from build123d import *

# Parameters (mm, degrees)
CUT_EXTRUDE1_DEPTH = 2.54
FILLET2_R          = 0.8128


with BuildPart() as part:
    # Sketch1 → Revolve1 (revolve)
    with BuildSketch(Plane.XY):
        Polygon((0, 5.842), (0, 12.7), (-6.35, 12.7), (-6.35, 0), (0, 0), (127, 0), (127, 5.842), align=None)
    revolve(axis=Axis((127, 0, 0), (-1, 0, 0)))

    # Sketch2 → Cut-Extrude1 (cut)
    with BuildSketch(Plane.ZY.offset(6.35)):
        Polygon((-2.54, 6.35), (-2.54, 2.54), (-6.35, 2.54), (-6.35, -2.54), (-2.54, -2.54), (-2.54, -6.122575092), (2.54, -6.122575092), (2.54, -2.54), (6.35, -2.54), (6.35, 2.54), (2.54, 2.54), (2.54, 6.35), align=None)
    extrude(amount=-CUT_EXTRUDE1_DEPTH, mode=Mode.SUBTRACT)

    # Fillet2
    fillet2_edges = [part.edges().sort_by_distance(p)[0] for p in [
        (-6.35, 6.35, 0),
        (-6.35, 4.445, -2.54),
        (-6.35, 2.54, -4.445),
        (-6.35, 0, -6.35),
        (-6.35, -2.54, -4.445),
        (-6.35, -4.331287546, -2.54),
        (-6.35, -6.122575092, 0),
        (-6.35, -4.331287546, 2.54),
        (-6.35, -2.54, 4.445),
        (-6.35, 0, 6.35),
        (-6.35, 2.54, 4.445),
        (-6.35, 4.445, 2.54),
    ]]
    fillet(fillet2_edges, radius=FILLET2_R)


solid = part.part
Geometry check sheet. Reference: the model listing, model coordinates, mm. Coordinates: 2 decimals unless noted, no trailing zeros. Loops run counter-clockwise (first coordinate to the right, second up) from the corner with the lowest first, then second, coordinate; pieces in that order, holes last. Notation, with made-up numbers: (-25.75, 46.5) - (14.25, 46.5) arc R26 cw to (14.25, 67.5) - close; hole circle Ø1 at (88.25, -3). An arc over 180 degrees is marked (long way). Use one line per item in the form item = value. Start each with the question number.
Item 1: Thickness scan on probe 1 along X at (y, z) = (-4.5, -0.5); probe 2 along Y at (x, z) = (37, 0); probe 3 along X at (y, z) = (4.25, 8.5). Record the ranges inside material, lowest first.
Item 2: Section check B-B, the plane y = 0. Enter the section's corners in (x, z), and give its area (3 significant figures).
Item 3: Mould release check, pull along Z, two halves, no side actions. Record for faces 1 (the face through (0, -5.5, 2.6)), 2 (the face through (62.611, -1.266, 5.703)), 3 (the face through (-3.81, 0, 0)): +Z half, -Z half, draft (parallel to the pull), parting line (faces both ways), or undercut.
Item 4: Section check C-C, the plane x = 78. Enter the section's corners in (y, z).
Item 5: Gauge pin test, flat ends, axial feed: pin 1 (1 mm diameter, centred on y = 3.5, z = 0, fed in from -X); pin 2 (6 mm diameter, centred on y = -7.5, z = -10, fed in from +X); pin 3 (1.9 mm diameter, centred on x = -4.5, y = -4.5, fed in from -Z). Record the tip position at first contact, or that the pin passes through.
Item 6: Section check D-D, the plane y = -9. Enter the section's corners in (x, z), and give its area (3 significant figures).
Item 7: Section check A-A, the plane z = 0. Enter the section's corners in (x, y).
Computed:
q1.probe_1 = -3.81 to 127
q1.probe_2 = -5.84 to 5.84
q1.probe_3 = -6.35 to 0
q2.outline = (-6.35, -12.7) - (0, -12.7) - (0, -5.84) - (127, -5.84) - (127, 5.84) - (0, 5.84) - (0, 12.7) - (-6.35, 12.7) - (-6.35, 7.16) arc R0.81 ccw to (-5.54, 6.35) - (-3.81, 6.35) - (-3.81, -6.35) - (-5.54, -6.35) arc R0.81 ccw to (-6.35, -7.16) - close
q2.area = 1,610 mm2
q3.face_1 = draft
q3.face_2 = parting line
q3.face_3 = undercut
q4.outline = circle Ø11.68 at (0, 0)
q5.pin_1 = -3.81
q5.pin_2 = 0
q5.pin_3 = -12.19
q6.outline = (-6.35, -8.96) - (0, -8.96) - (0, 8.96) - (-6.35, 8.96) - close
q6.area = 114 mm2
q7.outline = (-6.35, -12.7) - (0, -12.7) - (0, -5.84) - (127, -5.84) - (127, 5.84) - (0, 5.84) - (0, 12.7) - (-6.35, 12.7) - (-6.35, 7.16) arc R0.81 ccw to (-5.54, 6.35) - (-3.81, 6.35) - (-3.81, -6.12) - (-5.54, -6.12) arc R0.81 ccw to (-6.35, -6.94) - close
